Could you check a few things on this model? Use its own coordinates, in mm. Coordinates: 2 decimals unless noted, no trailing zeros. Order: outer loops, then holes, each group sorted by start corner. A loop starts at its lowest first (then second) coordinate and runs counter-clockwise, first axis right, second up. Notation, with made-up numbers: (13.5, -8.5) -> (47.5, -8.5) arc R13 ccw to (47.5, 5.5) -> close; hole circle Ø2 at (1.25, 53). An arc over 180 degrees is marked (long way). Use a Markdown table: item, result. Add a question column.
1) If we section it at B-B (y = 8.5): Give the number of separate pieces and of enclosed holes in the cut face, plus the area to 3 significant figures.
2) If we section it at D-D (x = -55): Write out the boundary of the cut face in (y, z), plus the area to 3 significant figures.
3) If I drill on L1, parallel to Z at x = -55.5, y = 1.5; L2, parallel to X at y = 8, z = 227.5; L3, parallel to Z at x = 69, y = 9, over which ranges is the centre line in solid material (lowest first)? Write a range as [from, to].
4) If we section it at A-A (x = 65): Write out the boundary of the cut face in (y, z), plus the area to 3 significant figures.
5) Will this pin go through, and if not, where does the flat tip stop? pin 1 Ø18 at (x, z) = (-55, 170) entering from -Y.
6) If we section it at C-C (x = 0): Write out the boundary of the cut face in (y, z), plus the area to 3 significant figures.
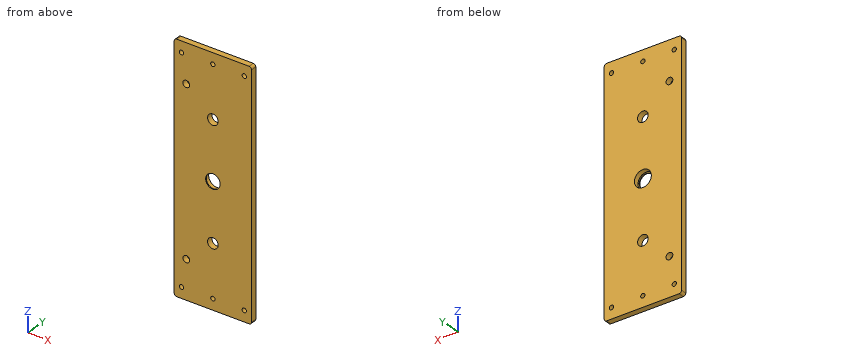
```python
from build123d import *

# Parameters (mm, degrees)
SKETCH1_W                    = 160
SKETCH1_H                    = 500
BOSS_EXTRUDE1_DEPTH          = 12
SKETCH2_R                    = 15
SKETCH2_R_2                  = 11
CUT_EXTRUDE1_DEPTH           = 12
SKETCH3_R                    = 17.5
CUT_EXTRUDE2_DEPTH           = 10
F_9_0_9_DIAMETER_HOLE1_D     = 9
F_9_0_9_DIAMETER_HOLE1_DEPTH = 13
F_9_0_9_DIAMETER_HOLE1_TIP   = 2.703872786
FILLET1_R                    = 5
SKETCH7_R                    = 7
CUT_EXTRUDE3_DEPTH           = 263.762249952


with BuildPart() as part:
    # Sketch1 → Boss-Extrude1 (new body)
    with BuildSketch(Plane(origin=(0, 0, 0), x_dir=(1, 0, 0), z_dir=(0, 1, 0))):
        Rectangle(SKETCH1_W, SKETCH1_H)
    extrude(amount=BOSS_EXTRUDE1_DEPTH)

    # Sketch2 → Cut-Extrude1 (cut)
    with BuildSketch(Plane(origin=(0, 12, 0), x_dir=(1, 0, 0), z_dir=(0, 1, 0))):
        with Locations(Location((0, 0, 0), (0, 0, 270))):
            Circle(SKETCH2_R)
        with Locations(Location((0, -120, 0), (0, 0, 270))):
            Circle(SKETCH2_R_2)
        with Locations(Location((0, 120, 0), (0, 0, 90))):
            Circle(SKETCH2_R_2)
    extrude(amount=-CUT_EXTRUDE1_DEPTH, mode=Mode.SUBTRACT)

    # Sketch3 → Cut-Extrude2 (cut)
    with BuildSketch(Plane(origin=(0, 12, 0), x_dir=(1, 0, 0), z_dir=(0, 1, 0))):
        with Locations(Location((0, 0, 0), (0, 0, 270))):
            Circle(SKETCH3_R)
    extrude(amount=-CUT_EXTRUDE2_DEPTH, mode=Mode.SUBTRACT)

    # Ø9.0 (9) Diameter Hole1
    with Locations(Plane(origin=(0, 12, 0), x_dir=(1, 0, 0), z_dir=(0, 1, 0))):
        with Locations((-65, 227.5), (0, 227.5), (65, 227.5), (-65, -227.5), (0, -227.5), (65, -227.5)):
            Hole(F_9_0_9_DIAMETER_HOLE1_D / 2, depth=F_9_0_9_DIAMETER_HOLE1_DEPTH)
            with Locations((0, 0, -(F_9_0_9_DIAMETER_HOLE1_DEPTH + F_9_0_9_DIAMETER_HOLE1_TIP / 2))):  # 118° drill point
                Cone(0, F_9_0_9_DIAMETER_HOLE1_D / 2, F_9_0_9_DIAMETER_HOLE1_TIP, mode=Mode.SUBTRACT)

    # Fillet1
    fillet1_edges = [part.edges().sort_by_distance(p)[0] for p in [
        (80, 6, 250),
        (-80, 6, 250),
        (-80, 6, -250),
        (80, 6, -250),
    ]]
    fillet(fillet1_edges, radius=FILLET1_R)

    # Sketch7 → Cut-Extrude3 (cut, through all)
    with BuildSketch(Plane.XZ):
        with Locations(Location((-55, 170, 0), (0, 0, 270))):
            Circle(SKETCH7_R)
        with Locations(Location((-55, -170, 0), (0, 0, 90))):
            Circle(SKETCH7_R)
    extrude(amount=-CUT_EXTRUDE3_DEPTH, mode=Mode.SUBTRACT)


solid = part.part
```
Answer sheet:
| question | item | result |
|---|---|---|
| 1 | separate pieces | 1 |
| 1 | enclosed holes | 11 |
| 1 | area | 77,600 mm2 |
| 2 | outline | (0, -250) -> (12, -250) -> (12, -177) -> (0, -177) -> close; (0, -163) -> (12, -163) -> (12, 163) -> (0, 163) -> close; (0, 177) -> (12, 177) -> (12, 250) -> (0, 250) -> close |
| 2 | area | 5,660 mm2 |
| 3 | L1 | [-250, -176.98], [-163.02, 163.02], [176.98, 250] |
| 3 | L2 | [-80, -69.5], [-60.5, -4.5], [4.5, 60.5], [69.5, 80] |
| 3 | L3 | [-250, -229.56], [-225.44, 225.44], [229.56, 250] |
| 4 | outline | (0, -250) -> (12, -250) -> (12, -232) -> (0, -232) -> close; (0, -223) -> (12, -223) -> (12, 223) -> (0, 223) -> close; (0, 232) -> (12, 232) -> (12, 250) -> (0, 250) -> close |
| 4 | area | 5,780 mm2 |
| 5 | pin 1 | y = 0 |
| 6 | outline | (0, -250) -> (12, -250) -> (12, -232) -> (0, -232) -> close; (0, -223) -> (12, -223) -> (12, -131) -> (0, -131) -> close; (0, -109) -> (12, -109) -> (12, -17.5) -> (2, -17.5) -> (2, -15) -> (0, -15) -> close; (0, 15) -> (2, 15) -> (2, 17.5) -> (12, 17.5) -> (12, 109) -> (0, 109) -> close; (0, 131) -> (12, 131) -> (12, 223) -> (0, 223) -> close; (0, 232) -> (12, 232) -> (12, 250) -> (0, 250) -> close |
| 6 | area | 4,850 mm2 |
